Here's how the part is built. I have some questions about the finished solid (model axes, mm). Round coordinates to 2 decimals unless told otherwise and drop trailing zeros. Write each loop counter-clockwise with the first axis right and the second up, starting at its lowest first coordinate (ties: lowest second). Pieces come first, ordered by that corner, then holes. Notation, with made-up numbers: (80, -39) -> (135, -39) arc R25 cw to (135, -18) -> close; hole circle Ø2 at (84.5, 28). An arc over 180 degrees is marked (long way). Answer in a Markdown table with one row per item.
from build123d import *

# Parameters (mm, degrees)
SKETCH_1_R         = 30
SKETCH_1_R_2       = 9.5
EXTRUDE_1_DEPTH    = 5
HOLE_WIZARD_M6_1_D = 7


with BuildPart() as part:
    # 草图1 → 凸台-拉伸1 (new body)
    with BuildSketch(Plane(origin=(0, 0, 0), x_dir=(1, 0, 0), z_dir=(0, 1, 0))):
        with Locations(Location((0, 0, 0), (0, 0, 270))):
            Circle(SKETCH_1_R)
        with Locations(Location((0, 0, 0), (0, 0, 270))):
            Circle(SKETCH_1_R_2, mode=Mode.SUBTRACT)
    extrude(amount=EXTRUDE_1_DEPTH)

    # M6 间隙孔1 (through all)
    with Locations(Plane(origin=(0, 5, 0), x_dir=(1, 0, 0), z_dir=(0, 1, 0))):
        with Locations((0, 16), (13.856406461, 8), (13.856406461, -8), (0, -16), (-13.856406461, -8), (-13.856406461, 8)):
            Hole(HOLE_WIZARD_M6_1_D / 2)


solid = part.part
1) I want a section at B-B, the plane y = 1.4. List the corners of the cut face in (x, z) for me, and give its area (3 significant figures).
Response:
| item | result |
|---|---|
| outline | circle Ø60 at (0, 0); hole circle Ø7 at (-13.86, -8); hole circle Ø7 at (-13.86, 8); hole circle Ø19 at (0, 0); hole circle Ø7 at (0, -16); hole circle Ø7 at (0, 16); hole circle Ø7 at (13.86, -8); hole circle Ø7 at (13.86, 8) |
| area | 2,310 mm^2 |
2) I want a section at A-A, the plane z = 0. List the corners of the cut face in (x, y) for me.
Response:
| item | result |
|---|---|
| outline | (-30, 0) -> (-9.5, 0) -> (-9.5, 5) -> (-30, 5) -> close; (9.5, 0) -> (30, 0) -> (30, 5) -> (9.5, 5) -> close |
3) I need wall thicknesses on line 1 (X direction, y = 1.15, z = 0); line 2 (X direction, y = 1.7, z = -10); line 3 (X direction, y = 0.3, z = 16.5). Which ranges of each line are inside material? Lowest first, please. Write a range as [from, to].
Response:
| item | result |
|---|---|
| line 1 | x = [-30, -9.5], [9.5, 30] |
| line 2 | x = [-28.28, -16.73], [-10.98, 10.98], [16.73, 28.28] |
| line 3 | x = [-25.05, -3.46], [3.46, 25.05] |
4) We'd pull the mould along X, two halves only. Please class faces 1 (the face through (7, 5, -7)), 2 (the face through (-3.233, 2.465, 17.341)), 3 (the face through (1.32, 2.46, -29.97)), 4 (the face through (-11.08, 2.47, -5.87)): +X half, -X half, draft (parallel to the pull), parting line (faces both ways), or undercut.
Response:
| item | result |
|---|---|
| face 1 | draft |
| face 2 | undercut |
| face 3 | parting line |
| face 4 | undercut |
5) I want a section at C-C, the plane x = 0. List the corners of the cut face in (y, z) for me, and give its area (3 significant figures).
Response:
| item | result |
|---|---|
| outline | (0, -30) -> (5, -30) -> (5, -19.5) -> (0, -19.5) -> close; (0, -12.5) -> (5, -12.5) -> (5, -9.5) -> (0, -9.5) -> close; (0, 9.5) -> (5, 9.5) -> (5, 12.5) -> (0, 12.5) -> close; (0, 19.5) -> (5, 19.5) -> (5, 30) -> (0, 30) -> close |
| area | 135 mm^2 |
6) I want a section at D-D, the plane z = 8. List the corners of the cut face in (x, y) for me, and give its area (3 significant figures).
Response:
| item | result |
|---|---|
| outline | (-28.91, 0) -> (-17.36, 0) -> (-17.36, 5) -> (-28.91, 5) -> close; (-10.36, 0) -> (-5.12, 0) -> (-5.12, 5) -> (-10.36, 5) -> close; (5.12, 0) -> (10.36, 0) -> (10.36, 5) -> (5.12, 5) -> close; (17.36, 0) -> (28.91, 0) -> (28.91, 5) -> (17.36, 5) -> close |
| area | 168 mm^2 |
7) For pin 1 (1 mm diameter, centred on x = 19, y = 2, fed in from +Z); pin 2 (1.5 mm diameter, centred on y = 1, z = -16, fed in from +X), each with a flat end and sliding along its axis, tell me the tip position at first contact or that it passes through.
Response:
| item | result |
|---|---|
| pin 1 | stops at z = 23.62 |
| pin 2 | stops at x = 25.83 |
